Verification items for the finished model (mm, model axes). A direction names the side the tool comes from. Give positions to 0.01 mm unless a question says otherwise; leave off trailing zeros. Order: outer loops, then holes, each group sorted by start corner. A loop starts at its lowest first (then second) coordinate and runs counter-clockwise, first axis right, second up.
(1) Sectioned sample at B-B on x = 65. Record the cut outline in (y, z).
(2) Mould release check, pull along X, two halves, no side actions. Record for faces 1 (the face through (91, 1, 11)), 2 (the face through (0, 0, 0)), 3 (the face through (60.152, 9, 20)), 4 (the face through (21, 4.5, 0)): pulls with the +X half, pulls with the -X half, needs draft (parallel to the pull), parting line crosses it, or undercut.
(3) Sectioned sample at A-A on z = 0. Record the cut outline in (x, y), plus the area to 3 significant figures.
(4) Gauge pin test, flat ends, axial feed: pin 1 (11 mm diameter, centred on x = 97, z = 3.5, fed in from +Y); pin 2 (7 mm diameter, centred on x = 21.34, z = 13.76, fed in from -Y); pin 3 (3.5 mm diameter, centred on x = 93, y = 2, fed in from -Z); pin 4 (5 mm diameter, centred on x = 76.5, z = -9.5, fed in from +Y). Record the tip position at first contact, or that the pin passes through.
(5) Access from +Z, -Z, +X, -X, +Y, -Y to the whole of each face (thin tool, end or side, straight path). Record for faces 5 (the face through (85, 4.5, 18)), 6 (the face through (103.986, -4.119, -20.297)), 7 (the face through (92, 1, -11)), 8 (the face through (81, -7, -4)).
(6) Scan lines: L1, parallel to X at y = 4.75, z = -0.5; L2, parallel to X at y = -4.25, z = 0; L3, parallel to Z at x = 25, y = -8. Record each from-to range of solid material in increasing order.
(7) Sectioned sample at C-C on y = 5.75. Record the cut outline in (x, z), plus the area to 3 significant figures.
(8) Sectioned sample at D-D on z = 12. Record the cut outline in (x, y).
```python
from build123d import *

# Parameters (mm, degrees)
BASE_OUTLINE_SKETCH_110X52_W      = 110
BASE_OUTLINE_SKETCH_110X52_H      = 52
BASE_BLOCK_25MM_DEPTH             = 12.5
SIDE_PROFILE_SKETCH_R             = 4.5
SIDE_PROFILE_CUT_THROUGH_75_DEPTH = 75
SIDE_PROFILE_CUT_8MM_DEPTH        = 8
SIDE_PROFILE_CUT_THROUGH_78_DEPTH = 78
SLOT_CUT_8MM_DEPTH                = 8
POCKET_CUT_15MM_DEPTH             = 15
END_FILLET_R20_R                  = 20


with BuildPart() as part:
    # Base Outline Sketch 110x52 → Base Block 25mm (new, symmetric)
    with BuildSketch(Plane(origin=(0, 0, 0), x_dir=(1, 0, 0), z_dir=(0, 1, 0))):
        with Locations((55, 0)):
            Rectangle(BASE_OUTLINE_SKETCH_110X52_W, BASE_OUTLINE_SKETCH_110X52_H)
    extrude(amount=BASE_BLOCK_25MM_DEPTH, both=True)

    # Side Profile Sketch → Side Profile Cut Through 75 (cut)
    with BuildSketch(Plane(origin=(0, 12.5, 0), x_dir=(1, 0, 0), z_dir=(0, 1, 0))):
        with Locations(Location((21.074107975, 13.849780556, 0), (0, 0, 270))):
            Circle(SIDE_PROFILE_SKETCH_R)
        with Locations(Location((21.343878228, -13.764722322, 0), (0, 0, 270))):
            Circle(SIDE_PROFILE_SKETCH_R)
    extrude(amount=-SIDE_PROFILE_CUT_THROUGH_75_DEPTH, mode=Mode.SUBTRACT)

    # Sketch2_6 → Side Profile Cut 8mm (cut)
    with BuildSketch(Plane(origin=(0, 12.5, 0), x_dir=(1, 0, 0), z_dir=(0, 1, 0))):
        with BuildLine():
            Line((9.587879583, 26), (34.858358674, 26))
            ThreePointArc((34.858358674, 26), (30, 0), (34.858358674, -26))
            Line((34.858358674, -26), (9.587879583, -26))
            ThreePointArc((9.587879583, -26), (6, 0), (9.587879583, 26))
        make_face()
    extrude(amount=-SIDE_PROFILE_CUT_8MM_DEPTH, mode=Mode.SUBTRACT)

    # Sketch2_9 → Side Profile Cut Through 78 (cut)
    with BuildSketch(Plane(origin=(0, 12.5, 0), x_dir=(1, 0, 0), z_dir=(0, 1, 0))):
        with BuildLine():
            Line((84, -4), (84, 4))
            Line((84, 4), (78.416407865, 4))
            ThreePointArc((78.416407865, 4), (51, 0), (78.416407865, -4))
            Line((78.416407865, -4), (84, -4))
        make_face()
    extrude(amount=-SIDE_PROFILE_CUT_THROUGH_78_DEPTH, mode=Mode.SUBTRACT)

    # Slot Sketch 22 → Slot Cut 8mm (cut)
    with BuildSketch(Plane(origin=(0, 12.5, 0), x_dir=(1, 0, 0), z_dir=(0, 1, 0))):
        with BuildLine():
            Line((60.152360051, 26), (60.152360051, 13.133940267))
            ThreePointArc((60.152360051, 13.133940267), (67.184589621, 13.828505638), (73.660254038, 11))
            Line((73.660254038, 11), (110, 11))
            Line((110, 11), (110, 26))
            Line((110, 26), (60.152360051, 26))
        make_face()
        with BuildLine():
            Line((73.660254038, -11), (110, -11))
            Line((110, -11), (110, -26))
            Line((110, -26), (60.152360051, -26))
            Line((60.152360051, -26), (60.152360051, -13.133940267))
            ThreePointArc((60.152360051, -13.133940267), (67.184589621, -13.828505638), (73.660254038, -11))
        make_face()
    extrude(amount=-SLOT_CUT_8MM_DEPTH, mode=Mode.SUBTRACT)

    # Pocket Sketch → Pocket Cut 15mm (cut)
    with BuildSketch(Plane(origin=(0, 12.5, 0), x_dir=(1, 0, 0), z_dir=(0, 1, 0))):
        with BuildLine():
            Line((110, 11), (73.660254038, 11))
            ThreePointArc((73.660254038, 11), (76.579928765, 7.86798893), (78.416407865, 4))
            Line((78.416407865, 4), (84, 4))
            Line((84, 4), (84, -4))
            Line((84, -4), (78.416407865, -4))
            ThreePointArc((78.416407865, -4), (76.579928765, -7.86798893), (73.660254038, -11))
            Line((73.660254038, -11), (110, -11))
            Line((110, -11), (110, 11))
        make_face()
    extrude(amount=-POCKET_CUT_15MM_DEPTH, mode=Mode.SUBTRACT)

    # End Fillet R20
    end_fillet_r20_edges = [part.edges().sort_by_distance(p)[0] for p in [
        (110, -4, -26),
        (110, -4, 26),
    ]]
    fillet(end_fillet_r20_edges, radius=END_FILLET_R20_R)


solid = part.part
```
Ans:
1. outline: (-12.5, -26) - (4.5, -26) - (4.5, -14) - (-12.5, -14) - close; (-12.5, 14) - (4.5, 14) - (4.5, 26) - (-12.5, 26) - close
2. face 1: needs draft
2. face 2: pulls with the -X half
2. face 3: pulls with the +X half
2. face 4: undercut
3. outline: (0, -12.5) - (51, -12.5) - (51, 12.5) - (30, 12.5) - (30, 4.5) - (6, 4.5) - (6, 12.5) - (0, 12.5) - close; (84, -12.5) - (110, -12.5) - (110, -2.5) - (84, -2.5) - close
3. area: 1,340 mm2
4. pin 1: stops at y = -2.5
4. pin 2: passes through
4. pin 3: stops at z = -25.96
4. pin 4: stops at y = 4.5
5. face 5: +Z, -Z, +X, +Y
5. face 6: -Z, +X, +Y, -Y
5. face 7: +X, +Y
5. face 8: +Y, -Y
6. L1: x = 0 to 6, 30 to 51.01
6. L2: x = 0 to 51, 84 to 110
6. L3: z = -26 to -16.05, -11.65 to 11.14, 16.39 to 26
7. outline: (0, -26) - (9.59, -26) arc R96 cw to (9.59, 26) - (0, 26) - close; (34.86, -26) - (60.15, -26) - (60.15, -13.13) arc R14 cw to (60.15, 13.13) - (60.15, 26) - (34.86, 26) arc R72 ccw to start
7. area: 1,680 mm2
8. outline: (0, -12.5) - (17.2, -12.5) - (17.2, 4.5) - (6.75, 4.5) - (6.75, 12.5) - (0, 12.5) - close; (25.48, -12.5) - (57.79, -12.5) - (57.79, 12.5) - (31.01, 12.5) - (31.01, 4.5) - (25.48, 4.5) - close; (72.21, -12.5) - (109.08, -12.5) - (109.08, 4.5) - (72.21, 4.5) - close
